```python
from build123d import *

# Parameters (mm, degrees)
SKETCH1_W                  = 250
SKETCH1_H                  = 100
BOSS_EXTRUDE1_DEPTH        = 4
F_14_0_14_DIAMETER_HOLE1_D = 14
FILLET1_R                  = 10


with BuildPart() as part:
    # Sketch1 → Boss-Extrude1 (new, symmetric)
    with BuildSketch(Plane.XY):
        Rectangle(SKETCH1_W, SKETCH1_H)
    extrude(amount=BOSS_EXTRUDE1_DEPTH, both=True)

    # Ø14.0 (14) Diameter Hole1 (through all)
    with Locations(Plane.XY.offset(4)):
        with Locations((-105, 37.5), (105, 37.5), (105, -37.5), (-105, -37.5)):
            Hole(F_14_0_14_DIAMETER_HOLE1_D / 2)

    # Fillet1
    fillet1_edges = [part.edges().sort_by_distance(p)[0] for p in [
        (-125, 50, 0),
        (125, 50, 0),
        (125, -50, 0),
        (-125, -50, 0),
    ]]
    fillet(fillet1_edges, radius=FILLET1_R)


solid = part.part
```
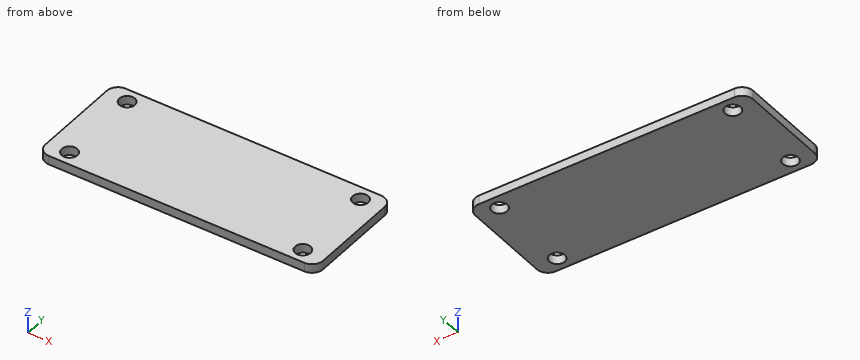
Work out the finished part from the listing and answer in its coordinate system (mm). Round coordinates to 2 decimals unless told otherwise and drop trailing zeros. Order: outer loops, then holes, each group sorted by start corner. A loop starts at its lowest first (then second) coordinate and runs counter-clockwise, first axis right, second up.
Q1. Find the intervals of material crossed by line 1 along Y through (x, z) = (105, -1.5); line 2 along X through (y, z) = (38, 1.5); line 3 along X through (y, z) = (-35.5, -0.5), in increasing order.
Solution:
line 1: y = -50 to -44.5, -30.5 to 30.5, 44.5 to 50
line 2: x = -125 to -111.98, -98.02 to 98.02, 111.98 to 125
line 3: x = -125 to -111.71, -98.29 to 98.29, 111.71 to 125
Q2. A cutting plane is placed at A-A, the plane y = -37.5. Determine the outline of the cut face in (x, z).
Solution:
outline: (-125, -4) - (-112, -4) - (-112, 4) - (-125, 4) - close; (-98, -4) - (98, -4) - (98, 4) - (-98, 4) - close; (112, -4) - (125, -4) - (125, 4) - (112, 4) - close
Q3. Given pin 1 Ø22.5 at (x, y) = (-105, 37.5) entering from +Z; pin 2 Ø11 at (x, y) = (105, 37.5) entering from -Z, each flat-ended and moving along its own axis, determine where each tip first touches the part or whether it passes through.
Solution:
pin 1: stops at z = 4
pin 2: passes through
Q4. A cutting plane is placed at C-C, the plane x = -109. Determine the outline of the cut face in (y, z), then the cut area to 3 significant figures.
Solution:
outline: (-50, -4) - (-43.24, -4) - (-43.24, 4) - (-50, 4) - close; (-31.76, -4) - (31.76, -4) - (31.76, 4) - (-31.76, 4) - close; (43.24, -4) - (50, -4) - (50, 4) - (43.24, 4) - close
area: 616 mm2
Q5. A cutting plane is placed at B-B, the plane z = -2.25. Determine the outline of the cut face in (x, y).
Solution:
outline: (-125, -40) arc R10 ccw to (-115, -50) - (115, -50) arc R10 ccw to (125, -40) - (125, 40) arc R10 ccw to (115, 50) - (-115, 50) arc R10 ccw to (-125, 40) - close; hole circle Ø14 at (-105, -37.5); hole circle Ø14 at (-105, 37.5); hole circle Ø14 at (105, -37.5); hole circle Ø14 at (105, 37.5)
